Design review of the part built by this model. Coordinates are the model's own, in mm. Face numbers are marked on the shaded views. A direction names the side the tool comes from. Coordinates: 2 decimals unless noted, no trailing zeros. Loops run counter-clockwise (first coordinate to the right, second up) from the corner with the lowest first, then second, coordinate; pieces in that order, holes last. Notation, with made-up numbers: (23, -30) - (46, -30) arc R19 ccw to (46, -4) - close; hole circle Ø1 at (80, 43). An arc over 180 degrees is marked (long way). Answer in a Markdown table with one row per item. Add a question column.
(1) To check wall thickness, follow L1, parallel to Y at x = -2.25, z = -8.5; L2, parallel to Y at x = 11.25, z = -34; L3, parallel to Z at x = 12, y = -1. State the ranges of each line that lie inside material, in increasing order. Write a range as [from, to].
(2) For the marked faces 4, 5 and 6, list the 3-axis set-ups (+Z, -Z, +X, -X, +Y, -Y) from which the entire face can be reached by the end or side of a thin tool; tool diameter is ignored.
(3) The part is to be moulded in two halves that separate along Z. For the marked faces 1, 2 and 3, say which applies: released by +Z, released by -Z, zero draft, split by the parting line, or undercut.
(4) Clearance check with flat-ended pins moving along their axes: pin 1 (3.5 mm diameter, centred on y = 1, z = -23.5, fed in from +X); pin 2 (1 mm diameter, centred on x = 16, y = -0.5, fed in from +Z); pin 3 (3.5 mm diameter, centred on y = -1.5, z = -7, fed in from +X); pin 4 (10 mm diameter, centred on y = 0, z = -8.5, fed in from -X). State where each tip first meets the part, or that it passes through.
(5) We need section A-A, the plane y = 0. Write out the cut boundary in (x, z), plus the area to 3 significant figures.
(6) We need section C-C, the plane y = -7. Write out the cut boundary in (x, z).
(7) We need section B-B, the plane x = 10.5. Write out the cut boundary in (y, z), plus the area to 3 significant figures.
(8) We need section D-D, the plane z = -35.5. Write out the cut boundary in (x, y).
from build123d import *

# Parameters (mm, degrees)
EXTRUDE_1_DEPTH              = 12.5
HOLE_WIZARD_M5_1_D           = 4.2
HOLE_WIZARD_M6_1_D           = 6.6
HOLE_WIZARD_M6_1_CBORE_D     = 11
HOLE_WIZARD_M6_1_CBORE_DEPTH = 6.4
CHAMFER_1_SIZE               = 2


with BuildPart() as part:
    # 草图1 → 凸台-拉伸1 (new, symmetric)
    with BuildSketch(Plane(origin=(0, 0, 0), x_dir=(1, 0, 0), z_dir=(0, 1, 0))):
        Polygon((0, 0), (0, 32), (21, 32), (21, 40), (-8, 40), (-8, 0), align=None)
    extrude(amount=EXTRUDE_1_DEPTH, both=True)

    # M5 螺纹孔1 (through all)
    with Locations(Plane.XY.offset(-32)):
        with Locations((10.5, 7), (10.5, -7)):
            Hole(HOLE_WIZARD_M5_1_D / 2)

    # M6 六角凹头螺钉的柱形沉头孔1 (through all)
    with Locations(Plane(origin=(0, 0, 0), x_dir=(0, 0, -1), z_dir=(1, 0, 0))):
        with Locations((8.5, 0), (23.5, 0)):
            CounterBoreHole(HOLE_WIZARD_M6_1_D / 2, HOLE_WIZARD_M6_1_CBORE_D / 2, HOLE_WIZARD_M6_1_CBORE_DEPTH)

    # 倒角1
    chamfer_1_edges = [part.edges().sort_by_distance(p)[0] for p in [
        (21, 12.5, -36),
        (-4, 12.5, 0),
        (21, -12.5, -36),
        (-4, -12.5, 0),
    ]]
    chamfer(chamfer_1_edges, length=CHAMFER_1_SIZE)


solid = part.part
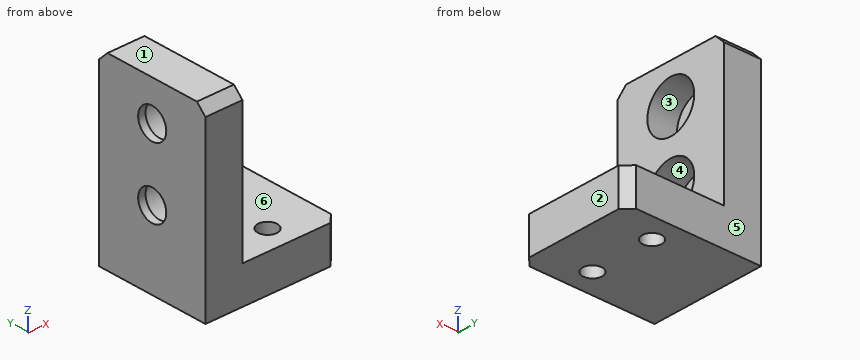
Responses:
| question | item | result |
|---|---|---|
| 1 | L1 | y = [-12.5, -5.5], [5.5, 12.5] |
| 1 | L2 | y = [-12.5, -8.96], [-5.04, 5.04], [8.96, 12.5] |
| 1 | L3 | z = [-40, -32] |
| 2 | face 4 | +X |
| 2 | face 5 | +Z, -Z, +X, -X, +Y |
| 2 | face 6 | +Z, +X, +Y, -Y |
| 3 | face 1 | released by +Z |
| 3 | face 2 | zero draft |
| 3 | face 3 | undercut |
| 4 | pin 1 | passes through |
| 4 | pin 2 | stops at z = -32 |
| 4 | pin 3 | stops at x = -6.4 |
| 4 | pin 4 | stops at x = -8 |
| 5 | outline | (-8, -40) - (21, -40) - (21, -32) - (0, -32) - (0, -29) - (-6.4, -29) - (-6.4, -26.8) - (-8, -26.8) - close; (-8, -20.2) - (-6.4, -20.2) - (-6.4, -18) - (0, -18) - (0, -14) - (-6.4, -14) - (-6.4, -11.8) - (-8, -11.8) - close; (-8, -5.2) - (-6.4, -5.2) - (-6.4, -3) - (0, -3) - (0, 0) - (-8, 0) - close |
| 5 | area | 326 mm2 |
| 6 | outline | (-8, -40) - (8.4, -40) - (8.4, -32) - (0, -32) - (0, 0) - (-8, 0) - close; (12.6, -40) - (21, -40) - (21, -32) - (12.6, -32) - close |
| 7 | outline | (-12.5, -40) - (-9.1, -40) - (-9.1, -32) - (-12.5, -32) - close; (-4.9, -40) - (4.9, -40) - (4.9, -32) - (-4.9, -32) - close; (9.1, -40) - (12.5, -40) - (12.5, -32) - (9.1, -32) - close |
| 7 | area | 133 mm2 |
| 8 | outline | (-8, -12.5) - (19, -12.5) - (21, -10.5) - (21, 10.5) - (19, 12.5) - (-8, 12.5) - close; hole circle Ø4.2 at (10.5, -7); hole circle Ø4.2 at (10.5, 7) |
